Geometry: final body of the model. Coordinates: model frame, mm. A direction names the side the tool comes from. Give positions to 0.01 mm unless a question says otherwise; leave off trailing zeros. Loops run counter-clockwise (first coordinate to the right, second up) from the corner with the lowest first, then second, coordinate; pieces in that order, holes last. Notation, with made-up numbers: M 47.5,4.5 L 54.5,4.5 A17 ccw 54.5,25.5 Z; hole C 59.25,64 d8. An arc over 180 degrees is marked long. Put each result on its own line as item: value.
```python
from build123d import *

# Parameters (mm, degrees)
SKETCH1_W           = 560
SKETCH1_H           = 560
SKETCH1_W_2         = 510
SKETCH1_H_2         = 510
BOSS_EXTRUDE1_DEPTH = 30
SKETCH2_R           = 6
BOSS_EXTRUDE2_DEPTH = 200
BOSS_EXTRUDE3_DEPTH = 20


with BuildPart() as part:
    # Sketch1 → Boss-Extrude1 (new body)
    with BuildSketch(Plane.XY):
        with Locations((280, 280)):
            Rectangle(SKETCH1_W, SKETCH1_H)
        with Locations((280, 280)):
            Rectangle(SKETCH1_W_2, SKETCH1_H_2, mode=Mode.SUBTRACT)
    extrude(amount=BOSS_EXTRUDE1_DEPTH)

    # Sketch2 → Boss-Extrude2 (add)
    with BuildSketch(Plane.XY.offset(30)):
        with Locations(Location((17, 543, 0), (0, 0, 180))):
            Circle(SKETCH2_R)
        with Locations(Location((17, 17, 0), (0, 0, 180))):
            Circle(SKETCH2_R)
        with Locations(Location((543, 17, 0), (0, 0, 180))):
            Circle(SKETCH2_R)
        with Locations(Location((543, 543, 0), (0, 0, 180))):
            Circle(SKETCH2_R)
        with Locations(Location((104, 543, 0), (0, 0, 180))):
            Circle(SKETCH2_R)
        with Locations(Location((104, 17, 0), (0, 0, 180))):
            Circle(SKETCH2_R)
        with Locations(Location((191, 543, 0), (0, 0, 180))):
            Circle(SKETCH2_R)
        with Locations(Location((191, 17, 0), (0, 0, 180))):
            Circle(SKETCH2_R)
        with Locations(Location((278, 543, 0), (0, 0, 180))):
            Circle(SKETCH2_R)
        with Locations(Location((278, 17, 0), (0, 0, 180))):
            Circle(SKETCH2_R)
        with Locations(Location((365, 543, 0), (0, 0, 180))):
            Circle(SKETCH2_R)
        with Locations(Location((365, 17, 0), (0, 0, 180))):
            Circle(SKETCH2_R)
        with Locations(Location((452, 543, 0), (0, 0, 180))):
            Circle(SKETCH2_R)
        with Locations(Location((452, 17, 0), (0, 0, 180))):
            Circle(SKETCH2_R)
        with Locations(Location((17, 104, 0), (0, 0, 180))):
            Circle(SKETCH2_R)
        with Locations(Location((543, 104, 0), (0, 0, 180))):
            Circle(SKETCH2_R)
        with Locations(Location((17, 191, 0), (0, 0, 180))):
            Circle(SKETCH2_R)
        with Locations(Location((543, 191, 0), (0, 0, 180))):
            Circle(SKETCH2_R)
        with Locations(Location((17, 278, 0), (0, 0, 180))):
            Circle(SKETCH2_R)
        with Locations(Location((543, 278, 0), (0, 0, 180))):
            Circle(SKETCH2_R)
        with Locations(Location((17, 365, 0), (0, 0, 180))):
            Circle(SKETCH2_R)
        with Locations(Location((543, 365, 0), (0, 0, 180))):
            Circle(SKETCH2_R)
        with Locations(Location((17, 452, 0), (0, 0, 180))):
            Circle(SKETCH2_R)
        with Locations(Location((543, 452, 0), (0, 0, 180))):
            Circle(SKETCH2_R)
    extrude(amount=BOSS_EXTRUDE2_DEPTH)

    # Sketch3 → Boss-Extrude3 (add)
    with BuildSketch(Plane.XY.offset(230)):
        with BuildLine():
            Line((7, 533), (7, 27))
            ThreePointArc((7, 27), (12.857864376, 12.857864376), (27, 7))
            Line((27, 7), (533, 7))
            ThreePointArc((533, 7), (547.142135624, 12.857864376), (553, 27))
            Line((553, 27), (553, 533))
            ThreePointArc((553, 533), (547.142135624, 547.142135624), (533, 553))
            Line((533, 553), (27, 553))
            ThreePointArc((27, 553), (12.857864376, 547.142135624), (7, 533))
        make_face()
        with BuildLine():
            Line((23, 532), (23, 28))
            ThreePointArc((23, 28), (24.464466094, 24.464466094), (28, 23))
            Line((28, 23), (532, 23))
            ThreePointArc((532, 23), (535.535533906, 24.464466094), (537, 28))
            Line((537, 28), (537, 532))
            ThreePointArc((537, 532), (535.535533906, 535.535533906), (532, 537))
            Line((532, 537), (28, 537))
            ThreePointArc((28, 537), (24.464466094, 535.535533906), (23, 532))
        make_face(mode=Mode.SUBTRACT)
    extrude(amount=BOSS_EXTRUDE3_DEPTH)


solid = part.part
```
Item 1: Mould query, pull axis Y, two halves, no side actions, for faces 1 (the flat face through (0, 276, 15)), 2 (the flat face through (284, 553, 240)), 3 (the flat face through (535, 276, 15)). Classes: pulls with the +Y half, pulls with the -Y half, needs draft (parallel to the pull), parting line crosses it, or undercut.
Output values:
face 1: needs draft
face 2: pulls with the +Y half
face 3: undercut
Item 2: Section A-A on y = 220.5. Output: boundary loops of the cut face in (x, z), then the cut area to 3 significant figures.
Output values:
outline: M 0,0 L 25,0 L 25,30 L 0,30 Z; M 7,230 L 23,230 L 23,250 L 7,250 Z; M 535,0 L 560,0 L 560,30 L 535,30 Z; M 537,230 L 553,230 L 553,250 L 537,250 Z
area: 2,140 mm²
Item 3: Pin query (flat end, axial travel): pin 1 Ø2.5 at (x, y) = (547, 547.5) entering from +Z; pin 2 Ø10 at (y, z) = (192.5, 241.5) entering from +X; pin 3 Ø10 at (x, z) = (336, 237) entering from +Y; pin 4 Ø10 at (y, z) = (318, 244.5) entering from -X. Return the tip coordinate at first contact, or that it passes through.
Output values:
pin 1: z = 250
pin 2: x = 553
pin 3: y = 553
pin 4: x = 7
Item 4: Line query: probe 1 along X at (y, z) = (290, 240); probe 2 along X at (y, z) = (534.5, 28). Output: solid intervals per line, ascending. Write a range as [from, to].
Output values:
probe 1: [7, 23], [537, 553]
probe 2: [0, 25], [535, 560]
Item 5: Set-up query: faces 4 (the flat face through (276, 535, 15)), 5 (the flat face through (284, 537, 240)), 6 (the flat face through (259, 544, 230)), 7 (the cylindrical face through (13.014, 547.297, 239.86)), 8 (the flat face through (276, 7, 240)). Return all of +Z, -Z, +X, -X, +Y, -Y with unobstructed straight access to the full face (end or side cutting, diameter ignored); none if empty.
Output values:
face 4: +Z, -Z
face 5: +Z
face 6: none
face 7: +Z, -X, +Y
face 8: +Z, +X, -X, -Y
Item 6: Section C-C on z = 204. Count the separate pieces of the cut face and the enclosed holes in it, then the cut area to 3 significant figures.
Output values:
separate pieces: 24
enclosed holes: 0
area: 2,710 mm²
